Could you check a few things on this model? Use its own coordinates, in mm. A direction names the side the tool comes from. Coordinates: 2 decimals unless noted, no trailing zeros. Write each loop counter-clockwise with the first axis right and the second up, starting at its lowest first coordinate (ties: lowest second). Pieces come first, ordered by that corner, then holes. Notation, with made-up numbers: M 32,34.25 L 66,34.25 A12 cw 66,45.25 Z; hole C 24.5,-18.5 d4. An arc over 180 degrees is marked long. Write item = value, one per line.
```python
from build123d import *


with BuildPart() as part:
    # 草图1 → 旋转1 (revolve)
    with BuildSketch(Plane.XY, mode=Mode.PRIVATE) as revolve_1_sk:
        Polygon((-425, 60), (425, 60), (425, 25), (433, 25), (433, 18), (561, 18), (561, 0), (-561, 0), (-561, 18), (-433, 18), (-433, 25), (-425, 25), align=None)
    revolve(revolve_1_sk.sketch.rotate(Axis((0, 0, 0), (1, 0, 0)), 90), axis=Axis((0, 0, 0), (1, 0, 0)))

    # 草图2 → M6 螺纹孔1 (revolve, cut)
    with BuildSketch(Plane(origin=(465.5, 18, 0), x_dir=(0, 0, 1), z_dir=(1, 0, 0))):
        Polygon((0, 0), (0, 5.443375673), (2.5, 4), (2.5, 0), align=None)
    hole_wizard_m6_1 = revolve(axis=Axis((465.5, 24.35, 0), (0, -1, 0)), mode=Mode.SUBTRACT)

    # 镜向1: M6 螺纹孔1 across plane
    add(hole_wizard_m6_1.mirror(Plane(origin=(0, 0, 0), x_dir=(0, 0, 1), z_dir=(1, 0, 0))), mode=Mode.SUBTRACT)


solid = part.part
```
Item 1: Imagine slicing it at A-A (y = 0). Write out the boundary of the cut face in (x, z).
Numbers:
outline = M -561,-18 L -433,-18 L -433,-25 L -425,-25 L -425,-60 L 425,-60 L 425,-25 L 433,-25 L 433,-18 L 561,-18 L 561,18 L 433,18 L 433,25 L 425,25 L 425,60 L -425,60 L -425,25 L -433,25 L -433,18 L -561,18 Z
Item 2: For faces 1 (the face through (425, 26, -1)), 2 (the face through (-425, -1, -26)), 3 (the face through (561, 0, 0)), which set-ups out of +Z, -Z, +X, -X, +Y, -Y let a thin tool reach every point of the face, with its end or its side?
Numbers:
face_1 = +X
face_2 = -X
face_3 = +Z, -Z, +X, +Y, -Y
Item 3: Imagine slicing it at D-D (x = -76.5). Write out the boundary of the cut face in (y, z), and give its area (3 significant figures).
Numbers:
outline = C 0,0 d120
area = 11,300 mm²
Item 4: If I drill on line 1 along X through (y, z) = (17, 0); line 2 along X through (y, z) = (-36, -16); line 3 along Z through (x, y) = (-465.5, 16.5), over which ranges is the centre line in solid material (lowest first)?
Numbers:
line_1 = -561 to -468, -463 to 463, 468 to 561
line_2 = -425 to 425
line_3 = -7.19 to -2.5, 2.5 to 7.19
Item 5: I'm going to push flat-ended pins straight in: P1, Ø5, axis at x = 384, z = -41, coming from the -Y side; P2, Ø8, axis at x = -347, y = 3.5, coming from the -Z side; P3, Ø6, axis at x = -266.5, y = -34, coming from the -Z side; P4, Ø6.5, axis at x = 465.5, z = 0, coming from the +Y side. Where does each tip first touch, or does it pass through?
Numbers:
P1 = -46.02
P2 = -60
P3 = -51.37
P4 = 18
Item 6: Imagine slicing it at C-C (z = -36). Write out the boundary of the cut face in (x, y), and give its area (3 significant figures).
Numbers:
outline = M -425,-48 L 425,-48 L 425,48 L -425,48 Z
area = 81,600 mm²
Item 7: Imagine slicing it at B-B (x = 483). Write out the boundary of the cut face in (y, z), and give its area (3 significant figures).
Numbers:
outline = C 0,0 d36
area = 1,020 mm²
